```python
from build123d import *

# Parameters (mm, degrees)
SKETCH1_R           = 12.5
SKETCH1_R_2         = 0.5
SKETCH1_W           = 6
SKETCH1_H           = 6
BOSS_EXTRUDE1_DEPTH = 2


with BuildPart() as part:
    # Sketch1 → Boss-Extrude1 (new body)
    with BuildSketch(Plane(origin=(0, 0, 0), x_dir=(1, 0, 0), z_dir=(0, 1, 0))):
        with Locations(Location((0, 0, 0), (0, 0, 270))):
            Circle(SKETCH1_R)
        with Locations(Location((-6, 6, 0), (0, 0, 270))):
            Circle(SKETCH1_R_2, mode=Mode.SUBTRACT)
        with Locations(Location((6, 6, 0), (0, 0, 270))):
            Circle(SKETCH1_R_2, mode=Mode.SUBTRACT)
        with Locations(Location((-6, -6, 0), (0, 0, 270))):
            Circle(SKETCH1_R_2, mode=Mode.SUBTRACT)
        with Locations(Location((6, -6, 0), (0, 0, 270))):
            Circle(SKETCH1_R_2, mode=Mode.SUBTRACT)
        Rectangle(SKETCH1_W, SKETCH1_H, mode=Mode.SUBTRACT)
    extrude(amount=BOSS_EXTRUDE1_DEPTH)


solid = part.part
```
Check sheet for the modelled part. Datum: model origin and axes. Units: mm. A direction names the side the tool comes from. Round coordinates to 2 decimals unless told otherwise and drop trailing zeros. Loops run counter-clockwise (first coordinate to the right, second up) from the corner with the lowest first, then second, coordinate; pieces in that order, holes last. Notation, with made-up numbers: (10.25, 21.5) - (58.25, 21.5) arc R16 ccw to (58.25, 28.5) - close; hole circle Ø8 at (0.5, 16.5). An arc over 180 degrees is marked (long way). Write item = value, one per line. Start each with the question number.
Q1. Release check for a two-part mould opening along X. For faces 1 (the face through (3.755, 0.986, 11.923)), 2 (the face through (0, 1, -3)), 3 (the face through (-5, 2, 0)) record: pulls with the +X half, pulls with the -X half, needs draft (parallel to the pull), parting line crosses it, or undercut.
Q2. Access from +Z, -Z, +X, -X, +Y, -Y to the whole of each face (thin tool, end or side, straight path). Record for faces 4 (the face through (-3, 1, 0)), 5 (the face through (-5, 0, 0)).
Q3. Section check B-B (y = 1.65). Record the boundary of the cut face in (x, z), plus the area to 3 significant figures.
Q4. Depth check by flat-ended pin: P1, Ø1, axis at y = 1.5, z = 4.5, coming from the +X side. Enter the tip coordinate at first touch or a pass-through.
Q5. Section check A-A (x = 0). Record the boundary of the cut face in (y, z).
Q6. Section check C-C (x = -6). Record the boundary of the cut face in (y, z), plus the area to 3 significant figures.
Q7. Thickness scan on L1, parallel to X at y = 0.85, z = 6; L2, parallel to Z at x = -0.25, y = 0.2; L3, parallel to Z at x = 1.5, y = 0.4. Record the ranges inside material, lowest first.
Q8. Section check D-D (z = 0.75). Record the boundary of the cut face in (x, y), plus the area to 3 significant figures.
Derived:
q1.face_1 = parting line crosses it
q1.face_2 = undercut
q1.face_3 = needs draft
q2.face_4 = +Y, -Y
q2.face_5 = +Z, -Z, +X, -X, -Y
q3.outline = circle Ø25 at (0, 0); hole circle Ø1 at (-6, -6); hole circle Ø1 at (-6, 6); hole (-3, -3) - (3, -3) - (3, 3) - (-3, 3) - close; hole circle Ø1 at (6, -6); hole circle Ø1 at (6, 6)
q3.area = 452 mm^2
q4.P1 = 11.84
q5.outline = (0, -12.5) - (2, -12.5) - (2, -3) - (0, -3) - close; (0, 3) - (2, 3) - (2, 12.5) - (0, 12.5) - close
q6.outline = (0, -10.97) - (2, -10.97) - (2, -6.5) - (0, -6.5) - close; (0, -5.5) - (2, -5.5) - (2, 5.5) - (0, 5.5) - close; (0, 6.5) - (2, 6.5) - (2, 10.97) - (0, 10.97) - close
q6.area = 39.9 mm^2
q7.L1 = -10.97 to -6.5, -5.5 to 5.5, 6.5 to 10.97
q7.L2 = -12.5 to -3, 3 to 12.5
q7.L3 = -12.41 to -3, 3 to 12.41
q8.outline = (-12.48, 0) - (-3, 0) - (-3, 2) - (-12.48, 2) - close; (3, 0) - (12.48, 0) - (12.48, 2) - (3, 2) - close
q8.area = 37.9 mm^2
